Build history of the part. All positions in model axes, mm. A direction names the side the tool comes from. Give positions to 0.01 mm unless a question says otherwise; leave off trailing zeros. Write each loop counter-clockwise with the first axis right and the second up, starting at its lowest first coordinate (ties: lowest second). Pieces come first, ordered by that corner, then holes. Notation, with made-up numbers: (-36.5, -6) -> (-0.5, -6) arc R7 cw to (-0.5, -1) -> close; hole circle Ø10 at (56, 71.25). An arc over 180 degrees is marked (long way). Put each result on its own line as item: value. Start each with the question number.
Item 1: Slice it at C-C, the plane y = -23. List the corners of the cut face in (x, z), plus the area to 3 significant figures.
Item 2: Slice it at B-B, the plane y = -12.25. List the corners of the cut face in (x, z).
Item 3: Drill centre lines: line 1 along Z through (x, y) = (27.5, 26); line 2 along Y through (x, z) = (25, 6); line 3 along Y through (x, z) = (18, 11). Where is each one in solid material? Low to high.
Item 4: Slice it at A-A, the plane x = -13. List the corners of the cut face in (y, z).
Item 5: Slice it at D-D, the plane z = -7. List the corners of the cut face in (x, y), plus the area to 3 significant figures.
Item 6: Two-plate mould, pull along X, no slides. Class faces 4 (the flat face through (39, -1, 19)), 5 (the flat face through (-1, 36.25, 0)), 6 (the conical face through (0.23, 20.01, 10.63)), 7 (the conical face through (27.18, 20.009, -11.293)): pulls with the +X half, pulls with the -X half, needs draft (parallel to the pull), parting line crosses it, or undercut.
Item 7: Flat gauge pins, fed straight in: pin 1 Ø4.5 at (x, y) = (17.5, -30.1) entering from -Z; pin 2 Ø6.5 at (x, z) = (0, 11) entering from -Y; pin 3 Ø4.5 at (x, z) = (0, -11) entering from +Y. Where does each tip first touch, or does it go through?
Item 8: Tool access for faces 1 (the flat face through (10, -33, 0)), 2 (the cylindrical face through (29, 29, -9)), 3 (the flat face through (-39, -1, -19)): list every direction of +Z, -Z, +X, -X, +Y, -Y with a clear straight run to the whole face (end or side of a thin tool).
```python
from build123d import *

# Parameters (mm, degrees)
SKETCH_1_W             = 80
SKETCH_1_H             = 72.5
SKETCH_1_R             = 20.75
EXTRUDE_1_DEPTH        = 20
SKETCH_2_W             = 20
SKETCH_2_H             = 6.318622164
CUT_EXTRUDE_1_DEPTH    = 68.186773252
HOLE_WIZARD_M6_1_D     = 5
HOLE_WIZARD_M6_2_D     = 5
HOLE_WIZARD_M6_2_DEPTH = 15
HOLE_WIZARD_M6_2_TIP   = 1.502151548
CHAMFER_1_SIZE         = 2


with BuildPart() as part:
    # 草图1 → 凸台-拉伸1 (new, symmetric)
    with BuildSketch(Plane.XY):
        Rectangle(SKETCH_1_W, SKETCH_1_H)
        with Locations((0, -11.75)):
            Circle(SKETCH_1_R, mode=Mode.SUBTRACT)
    extrude(amount=EXTRUDE_1_DEPTH, both=True)

    # 草图2 → 切除-拉伸1 (cut, through all)
    with BuildSketch(Plane.XY.offset(20)):
        with Locations((0, -33.090688918)):
            Rectangle(SKETCH_2_W, SKETCH_2_H)
    extrude(amount=-CUT_EXTRUDE_1_DEPTH, mode=Mode.SUBTRACT)

    # M6 螺纹孔1 (through all)
    with Locations(Plane(origin=(0, 0, -20), x_dir=(-1, 0, 0), z_dir=(0, 0, -1))):
        with Locations((-17.5, 5.603571071), (17.5, 5.603571071), (17.5, -30.103571071), (-17.5, -30.103571071), (-25, -12.25), (25, -12.25)):
            Hole(HOLE_WIZARD_M6_1_D / 2)

    # M6 螺纹孔2
    with Locations(Plane(origin=(0, 36.25, 0), x_dir=(1, 0, 0), z_dir=(0, 1, 0))):
        with Locations((-27.5, 11), (-27.5, -11), (27.5, -11), (27.5, 11), (0, 11), (0, -11)):
            Hole(HOLE_WIZARD_M6_2_D / 2, depth=HOLE_WIZARD_M6_2_DEPTH)
            with Locations((0, 0, -(HOLE_WIZARD_M6_2_DEPTH + HOLE_WIZARD_M6_2_TIP / 2))):  # 118° drill point
                Cone(0, HOLE_WIZARD_M6_2_D / 2, HOLE_WIZARD_M6_2_TIP, mode=Mode.SUBTRACT)

    # 倒角1
    chamfer_1_edges = [part.edges().sort_by_distance(p)[0] for p in [
        (-40, 0, 20),
        (40, 0, 20),
        (-40, 0, -20),
        (40, 0, -20),
    ]]
    chamfer(chamfer_1_edges, length=CHAMFER_1_SIZE)


solid = part.part
```
Values follow:
1. outline: (-40, -18) -> (-38, -20) -> (-17.44, -20) -> (-17.44, 20) -> (-38, 20) -> (-40, 18) -> close; (17.44, -20) -> (38, -20) -> (40, -18) -> (40, 18) -> (38, 20) -> (17.44, 20) -> close
1. area: 1,800 mm2
2. outline: (-40, -18) -> (-38, -20) -> (-27.5, -20) -> (-27.5, 20) -> (-38, 20) -> (-40, 18) -> close; (-22.5, -20) -> (-20.74, -20) -> (-20.74, 20) -> (-22.5, 20) -> close; (20.74, -20) -> (22.5, -20) -> (22.5, 20) -> (20.74, 20) -> close; (27.5, -20) -> (38, -20) -> (40, -18) -> (40, 18) -> (38, 20) -> (27.5, 20) -> close
3. line 1: -20 to -13.5, -8.5 to 8.5, 13.5 to 20
3. line 2: -36.25 to -14.75, -9.75 to 36.25
3. line 3: -36.25 to -32.55, -27.65 to -22.07, -1.43 to 3.15, 8.05 to 36.25
4. outline: (-36.25, -20) -> (-27.92, -20) -> (-27.92, 20) -> (-36.25, 20) -> close; (4.42, -20) -> (36.25, -20) -> (36.25, 20) -> (4.42, 20) -> close
5. outline: (-40, -36.25) -> (-10, -36.25) -> (-10, -29.93) arc R20.75 cw (long way) to (10, -29.93) -> (10, -36.25) -> (40, -36.25) -> (40, 36.25) -> (-40, 36.25) -> close; hole circle Ø5 at (-25, -12.25); hole circle Ø5 at (-17.5, -30.1); hole circle Ø5 at (-17.5, 5.6); hole circle Ø5 at (17.5, -30.1); hole circle Ø5 at (17.5, 5.6); hole circle Ø5 at (25, -12.25)
5. area: 4,240 mm2
6. face 4: pulls with the +X half
6. face 5: needs draft
6. face 6: undercut
6. face 7: undercut
7. pin 1: through
7. pin 2: y = 8.74
7. pin 3: y = 21.1
8. face 1: +Z, -Z, -Y
8. face 2: +Y
8. face 3: -Z, -X, +Y, -Y
